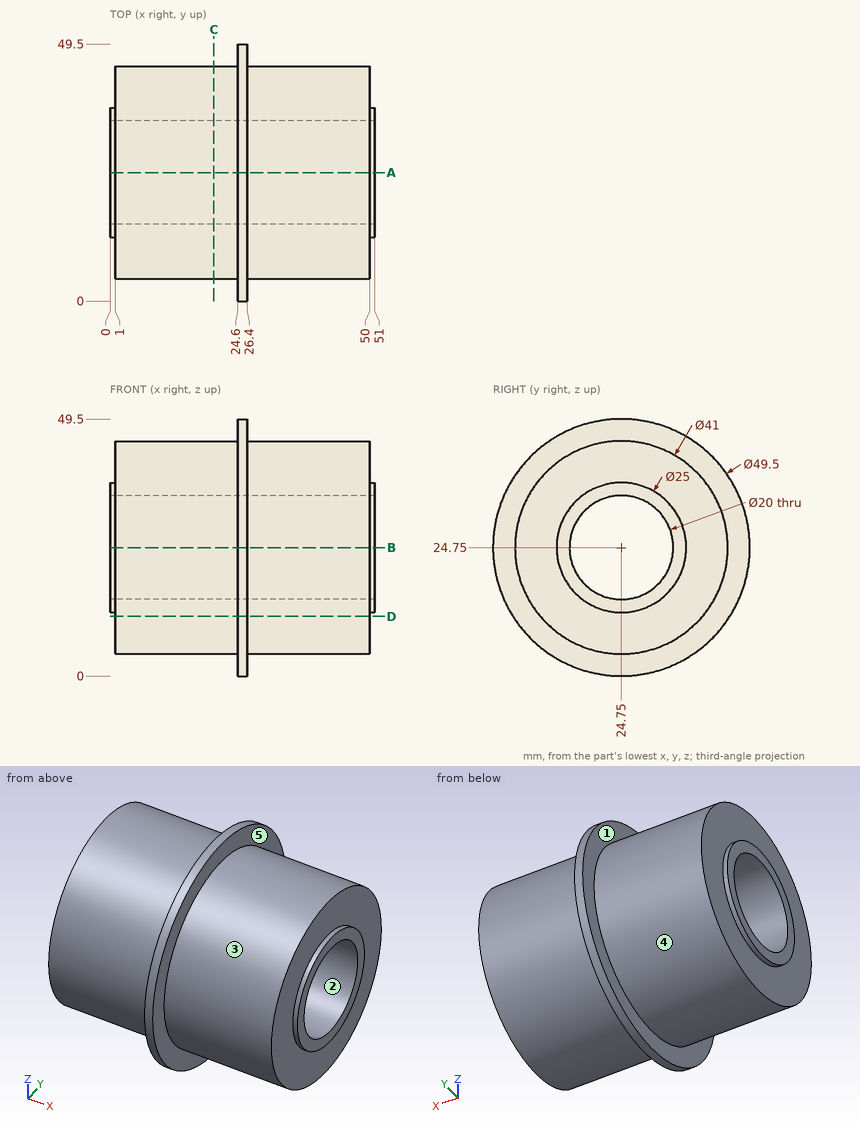
For this review, use the dimensioned drawing (mm, ordinates from the lowest corner) and the shaded views. A direction names the side the tool comes from. Give positions to 0.01 mm unless a question says otherwise; leave off trailing zeros. Order: outer loops, then holes, each group sorted by start corner. A loop starts at its lowest first (then second) coordinate and runs counter-clockwise, first axis right, second up. Notation, with made-up numbers: (-31.75, 62) - (-15.75, 62) arc R9 cw to (-15.75, 75) - close; hole circle Ø5 at (57, 35). An arc over 180 degrees is marked (long way). Use CSV: the item, a comma, the result in double quotes. Start each with the question number.
Q1. Draft analysis for pull direction Z (two halves, no side actions). For the marked faces 1, 2 and 3, state which applies: pulls with the +Z half, pulls with the -Z half, needs draft (parallel to the pull), parting line crosses it, or undercut.
Q2. For P1, Ø1.5, axis at x = 17, y = 18.5, coming from the -Z side; P2, Ø6, axis at y = 36, z = 10, coming from the -X side; P3, Ø6, axis at x = 13.5, z = 42.5, coming from the -Y side; P4, Ø1.5, axis at y = 32, z = 29, coming from the +X side, all flat-tipped, find the tip position at first contact; note any pin that passes through.
Q3. Take a section at C-C (x = 20). State the section outline as (y, z) points.
Q4. Take a section at D-D (z = 11.5). State the section outline as (x, y) points, and give its area (3 significant figures).
Q5. For line 1 (Y direction, x = 15, z = 24.75); line 2 (X direction, y = 29.5, z = 41); line 3 (Z direction, x = 42.5, y = 18), list the stretches that pass through material, from the lowest coordinate up.
Q6. Machinability: for the marked faces 4 and 5, which of the approach directions +Z, -Z, +X, -X, +Y, -Y give a long, thin tool a straight path to every point of the face, cutting with its end or side? Answer none if there is none.
Q7. Take a section at A-A (y = 24.75). State the section outline as (x, z) points, and give its area (3 significant figures).
Calculated:
1,face 1,"needs draft"
1,face 2,"undercut"
1,face 3,"parting line crosses it"
2,P1,"stops at z = 5"
2,P2,"stops at x = 1"
2,P3,"stops at y = 10.51"
2,P4,"passes through"
3,outline,"circle Ø41 at (24.75, 24.75); hole circle Ø20 at (24.75, 24.75)"
4,outline,"(1, 9.11) - (24.6, 9.11) - (24.6, 3.85) - (26.4, 3.85) - (26.4, 9.11) - (50, 9.11) - (50, 40.39) - (26.4, 40.39) - (26.4, 45.65) - (24.6, 45.65) - (24.6, 40.39) - (1, 40.39) - close"
4,area,"1,550 mm²"
5,line 1,"y = 4.25 to 14.75, 34.75 to 45.25"
5,line 2,"x = 1 to 50"
5,line 3,"z = 5.39 to 17.37, 32.13 to 44.11"
6,face 4,"-X"
6,face 5,"+X"
7,outline,"(0, 12.25) - (1, 12.25) - (1, 4.25) - (24.6, 4.25) - (24.6, 0) - (26.4, 0) - (26.4, 4.25) - (50, 4.25) - (50, 12.25) - (51, 12.25) - (51, 14.75) - (0, 14.75) - close; (0, 34.75) - (51, 34.75) - (51, 37.25) - (50, 37.25) - (50, 45.25) - (26.4, 45.25) - (26.4, 49.5) - (24.6, 49.5) - (24.6, 45.25) - (1, 45.25) - (1, 37.25) - (0, 37.25) - close"
7,area,"1,050 mm²"
